```python
from build123d import *

# Parameters (mm, degrees)
STRUCTURAL_MEMBER1_DEPTH = 1300


with BuildPart() as part:
    # Sketch1 → Structural Member1 (new body)
    with BuildSketch(Plane.YZ.offset(-650)):
        with BuildLine():
            Line((0, 0), (0, -120))
            Line((0, -120), (-53, -120))
            Line((-53, -120), (-53, -117.44744403))
            ThreePointArc((-53, -117.44744403), (-51.836536401, -114.427920086), (-48.947766736, -112.969776674))
            Line((-48.947766736, -112.969776674), (-13.604466529, -109.435446653))
            ThreePointArc((-13.604466529, -109.435446653), (-7.826927198, -106.519159828), (-5.5, -100.480111941))
            Line((-5.5, -100.480111941), (-5.5, -19.519888059))
            ThreePointArc((-5.5, -19.519888059), (-7.826927198, -13.480840172), (-13.604466529, -10.564553347))
            Line((-13.604466529, -10.564553347), (-48.947766736, -7.030223326))
            ThreePointArc((-48.947766736, -7.030223326), (-51.836536401, -5.572079914), (-53, -2.55255597))
            Line((-53, -2.55255597), (-53, 0))
            Line((-53, 0), (0, 0))
        make_face()
    extrude(amount=STRUCTURAL_MEMBER1_DEPTH)


solid = part.part
```
Verification items for the finished model (mm, model axes). A direction names the side the tool comes from. Coordinates: 2 decimals unless noted, no trailing zeros. Order: outer loops, then holes, each group sorted by start corner. A loop starts at its lowest first (then second) coordinate and runs counter-clockwise, first axis right, second up. Notation, with made-up numbers: (87, 41.5) -> (95, 41.5) arc R11 ccw to (95, 47.5) -> close; hole circle Ø1 at (-35, 17.25). An arc over 180 degrees is marked (long way). Put each result on its own line as item: value. Start each with the question number.
1) Material ranges on L1, parallel to Y at x = -242, z = -61; L2, parallel to Z at x = 432, y = -6.5; L3, parallel to Z at x = -68.5, y = -23 (3 decimals), recorded low to high.
2) Cross-section at A-A (y = -22.5). Enter the section's corners in (x, z) (3 decimals).
3) Release check for a two-part mould opening along Z. For faces 1 (the flat face through (-9, -5.5, -61)), 2 (the flat face through (-9, 0, -59)), 3 (the flat face through (-9, -26, -120)) record: pulls with the +Z half, pulls with the -Z half, needs draft (parallel to the pull), parting line crosses it, or undercut.
4) Cross-section at B-B (x = 401). Enter the section's corners in (y, z).
5) Go/stop test with flat-tipped pins: pin 1 (24.5 mm diameter, centred on x = -96, z = -59, fed in from -Y); pin 2 (12 mm diameter, centred on x = 467.5, y = -33, fed in from +Z). Record where each tip stops, or that it passes through.
6) Cross-section at C-C (z = -30). Enter the section's corners in (x, y).
7) Tool access check on faces 4 (the flat face through (-9.1, -31.03, -8.82)), 5 (the flat face through (-9, -27, 0)). Record the directions out of +Z, -Z, +X, -X, +Y, -Y that give a thin tool (end or side, any length) a straight path to the whole face; none if there is none.
Geometry check:
1. L1: y = -5.5 to 0
1. L2: z = -120 to -104.6, -15.4 to 0
1. L3: z = -120 to -110.375, -9.625 to 0
2. outline: (-650, -120) -> (650, -120) -> (650, -110.325) -> (-650, -110.325) -> close; (-650, -9.675) -> (650, -9.675) -> (650, 0) -> (-650, 0) -> close
3. face 1: undercut
3. face 2: needs draft
3. face 3: pulls with the -Z half
4. outline: (-53, -120) -> (0, -120) -> (0, 0) -> (-53, 0) -> (-53, -2.55) arc R4.5 ccw to (-48.95, -7.03) -> (-13.6, -10.56) arc R9 cw to (-5.5, -19.52) -> (-5.5, -100.48) arc R9 cw to (-13.6, -109.44) -> (-48.95, -112.97) arc R4.5 ccw to (-53, -117.45) -> close
5. pin 1: stops at y = -5.5
5. pin 2: stops at z = 0
6. outline: (-650, -5.5) -> (650, -5.5) -> (650, 0) -> (-650, 0) -> close
7. face 4: +X, -X, -Y
7. face 5: +Z, +X, -X, +Y, -Y
